from build123d import *

# Parameters (mm, degrees)
SKETCH1_R           = 32.5
SKETCH1_R_2         = 25
BOSS_EXTRUDE1_DEPTH = 3.5
SKETCH2_R           = 31.5
SKETCH2_R_2         = 26.25
CUT_EXTRUDE1_DEPTH  = 0.2
FILLET1_R           = 0.5


with BuildPart() as part:
    # Sketch1 → Boss-Extrude1 (new, symmetric)
    with BuildSketch(Plane.XY):
        Circle(SKETCH1_R)
        Circle(SKETCH1_R_2, mode=Mode.SUBTRACT)
    extrude(amount=BOSS_EXTRUDE1_DEPTH, both=True)

    # Sketch2 → Cut-Extrude1 (cut)
    with BuildSketch(Plane.XY.offset(3.5)):
        Circle(SKETCH2_R)
        Circle(SKETCH2_R_2, mode=Mode.SUBTRACT)
    cut_extrude1 = extrude(amount=-CUT_EXTRUDE1_DEPTH, mode=Mode.SUBTRACT)

    # Mirror1: Cut-Extrude1 across plane
    add(cut_extrude1.mirror(Plane.XY), mode=Mode.SUBTRACT)

    # Fillet1
    fillet1_edges = [part.edges().sort_by_distance(p)[0] for p in [
        (-32.5, 0, -3.5),
        (-32.5, 0, 3.5),
        (-25, 0, -3.5),
        (-25, 0, 3.5),
    ]]
    fillet(fillet1_edges, radius=FILLET1_R)


solid = part.part
Check sheet for the modelled part. Datum: model origin and axes. Units: mm. A direction names the side the tool comes from. Round coordinates to 2 decimals unless told otherwise and drop trailing zeros. Loops run counter-clockwise (first coordinate to the right, second up) from the corner with the lowest first, then second, coordinate; pieces in that order, holes last. Notation, with made-up numbers: (50.5, 83.5) - (70.5, 83.5) arc R25 cw to (70.5, 101.5) - close; hole circle Ø3 at (68.5, 15.25). An arc over 180 degrees is marked (long way). Answer as CSV lines item,"result". Start each with the question number.
Item 1: Section check C-C (z = 1.5). Record the boundary of the cut face in (x, y), and give its area (3 significant figures).
Item 2: Release check for a two-part mould opening along X. For faces 1 (the cylindrical face through (31, 9.76, 0.04)), 2 (the flat face through (23.6, -21.2, -3.5)), 3 (the flat face through (-7, 26, 3.3)), 4 (the cylindrical face through (23.846, 7.509, -0.042)) record: +X half, -X half, draft (parallel to the pull), parting line (faces both ways), or undercut.
Item 3: Scan lines: line 1 (Y direction, x = 0, z = 3.4); line 2 (Y direction, x = 0, z = -3.35); line 3 (Y direction, x = 0, z = 1.55). Record each from-to range of solid material in increasing order. Write a range as [from, to].
Item 4: Depth check by flat-ended pin: P1, Ø1, axis at y = -21.5, z = -2.5, coming from the +X side; P2, Ø1, axis at y = -17.5, z = 1.5, coming from the +X side. Enter the tip coordinate at first touch or a pass-through.
Item 5: Set-up check for faces 5 (the flat face through (23.6, -21.2, 3.5)), 6 (the flat face through (-7, 26, -3.3)): record each of +Z, -Z, +X, -X, +Y, -Y from which the full face is reachable in a straight line by a thin tool's end or side.
Report:
1,outline,"circle Ø65 at (0, 0); hole circle Ø50 at (0, 0)"
1,area,"1,350 mm2"
2,face 1,"parting line"
2,face 2,"draft"
2,face 3,"undercut"
2,face 4,"undercut"
3,line 1,"y = [-32.3, -31.5], [-26.25, -25.2], [25.2, 26.25], [31.5, 32.3]"
3,line 2,"y = [-32.36, -31.5], [-26.25, -25.14], [25.14, 26.25], [31.5, 32.36]"
3,line 3,"y = [-32.5, -25], [25, 32.5]"
4,P1,"stops at x = 24.8"
4,P2,"stops at x = 27.7"
5,face 5,"+Z, +X, -X, +Y, -Y"
5,face 6,"-Z"
